from build123d import *

# Parameters (mm, degrees)
SKETCH_2_R          = 28
CUT_EXTRUDE_1_DEPTH = 185
SKETCH_4_R          = 34
SKETCH_3_R          = 28
CUT_EXTRUDE_2_DEPTH = 50


with BuildPart() as part:
    # 草图1 → 旋转1 (revolve)
    with BuildSketch(Plane.XY, mode=Mode.PRIVATE) as revolve_1_sk:
        Polygon((0, 92.5), (0, -92.5), (31, -92.5), (34, -73.5), (32, -73.5), (32, -54.5), (34, -44.5), (32, -44.5), (32, -25.5), (34, -15.5), (32, -15.5), (32, 3.5), (34, 13.5), (32, 13.5), (32, 32.5), (34, 42.5), (32, 42.5), (32, 52.5), (38, 62.5), (38, 90.5), (36, 92.5), align=None)
    revolve(revolve_1_sk.sketch.rotate(Axis((0, 92.5, 0), (0, -1, 0)), 90), axis=Axis((0, 92.5, 0), (0, -1, 0)))

    # 草图2 → 切除-拉伸1 (cut)
    with BuildSketch(Plane(origin=(0, 92.5, 0), x_dir=(1, 0, 0), z_dir=(0, 1, 0))):
        with Locations(Location((0, 0, 0), (0, 0, 270))):
            Circle(SKETCH_2_R)
    extrude(amount=-CUT_EXTRUDE_1_DEPTH, mode=Mode.SUBTRACT)

    # 草图4 → 切除-放样1 section 0
    with BuildSketch(Plane(origin=(0, 92.5, 0), x_dir=(1, 0, 0), z_dir=(0, 1, 0))):
        Circle(SKETCH_4_R)
    # 草图3 → 切除-放样1 section 1
    with BuildSketch(Plane(origin=(0, 62.5, 0), x_dir=(-1, 0, 0), z_dir=(0, 1, 0))):
        Circle(SKETCH_3_R)
    loft(mode=Mode.SUBTRACT)

    # 草图5 → 切除-拉伸2 (cut, symmetric)
    with BuildSketch(Plane(origin=(0, 0, 0), x_dir=(0, 0, -1), z_dir=(1, 0, 0))):
        Polygon((-38, 77.5), (38, 92.5), (-38, 92.5), align=None)
    extrude(amount=CUT_EXTRUDE_2_DEPTH, both=True, mode=Mode.SUBTRACT)


solid = part.part
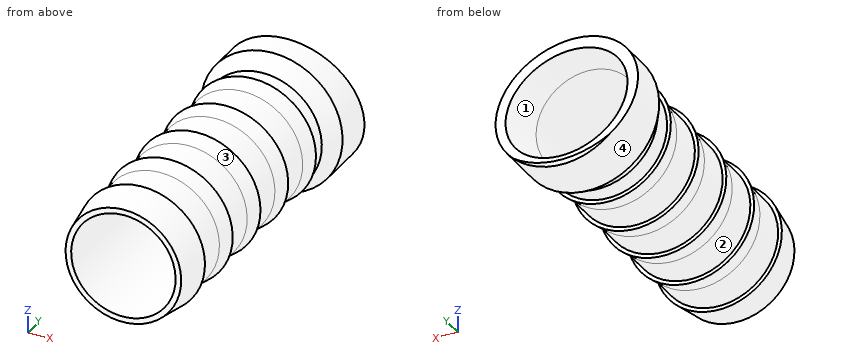
Design review of the part built by this model. Coordinates are the model's own, in mm. Face numbers are marked on the shaded views. A direction names the side the tool comes from. Coordinates: 2 decimals unless noted, no trailing zeros. Write each loop counter-clockwise with the first axis right and the second up, starting at its lowest first coordinate (ties: lowest second). Pieces come first, ordered by that corner, then holes. Notation, with made-up numbers: (82.5, -28) - (128.5, -28) arc R15 cw to (128.5, -16) - close; hole circle Ø9 at (4.5, -28.75). An arc over 180 degrees is marked (long way). Use one line per item in the form item = value.
Q1. Consider section A-A (y = 60). Write out the cut boundary in (x, z).
Taken from the geometry:
outline = circle Ø73 at (0, 0); hole circle Ø56 at (0, 0)
Q2. Insertion check: pin 1 Ø12 at (y, z) = (5.5, -23.5) entering from +X; pin 2 Ø12 at (x, y) = (-3, -70.5) entering from +Z; pin 3 Ø20.5 at (x, z) = (14.5, 2) entering from +Y; pin 4 Ø10 at (x, y) = (17.5, -28) entering from +Z. Each pin has a flat end and moves straight along its axis. Give the tip position at first contact, or say it passes through.
Taken from the geometry:
pin_1 = 27.52
pin_2 = 34
pin_3 = through
pin_4 = 29.46
Q3. For probe 1 along Z at (x, y) = (0.5, 32); probe 2 along X at (y, z) = (-7, 21.5), list the stretches that pass through material, from the lowest coordinate up.
Taken from the geometry:
probe_1 = -32 to -28, 28 to 32
probe_2 = -23.7 to -17.94, 17.94 to 23.7
Q4. The part is to be moulded in two halves that separate along X. For the marked faces 1 and 2, say which applies: +X half, -X half, draft (parallel to the pull), parting line (faces both ways), or undercut.
Taken from the geometry:
face_1 = undercut
face_2 = parting line
Q5. Machinability: for the marked faces 3 and 4, which of the approach directions +Z, -Z, +X, -X, +Y, -Y give a long, thin tool a straight path to every point of the face, cutting with its end or side? Answer none if there is none.
Taken from the geometry:
face_3 = none
face_4 = +Y, -Y
